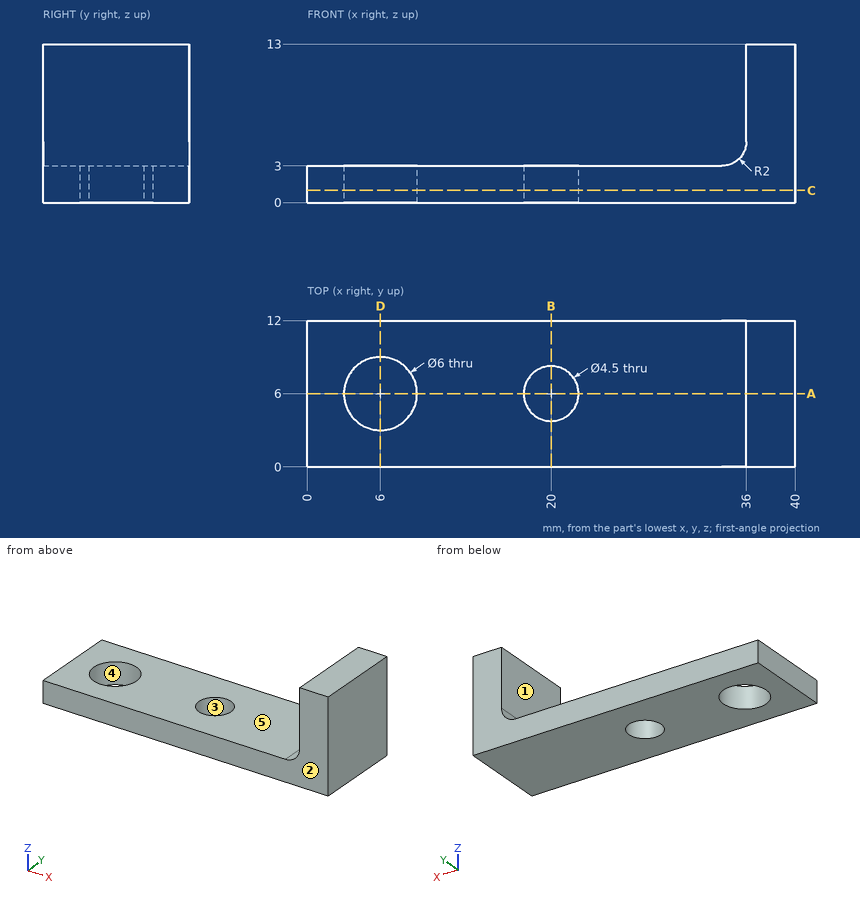
Check sheet for the drawn part. Datum: minimum x, y, z corner. Units: mm. A direction names the side the tool comes from. Coordinates: 2 decimals unless noted, no trailing zeros. Order: outer loops, then holes, each group sorted by start corner. A loop starts at its lowest first (then second) coordinate and runs counter-clockwise, first axis right, second up. Notation, with made-up numbers: M 11,82 L 52,82 A14 cw 52,102 Z; hole C 26,17.25 d10. An arc over 180 degrees is marked long. One line per item, written item: value. Start each with the question number.
Item 1: Sectioned sample at C-C (z = 1). Enter the section's corners in (x, y), then the cut area to 3 significant figures.
Item 2: Gauge pin test, flat ends, axial feed: pin 1 (5 mm diameter, centred on x = 6, y = 6, fed in from -Z); pin 2 (3.5 mm diameter, centred on x = 22.5, y = 7, fed in from +Z); pin 3 (3 mm diameter, centred on x = 27, y = 7.5, fed in from -Z); pin 4 (6.5 mm diameter, centred on y = 8.5, z = 8, fed in from -X). Record the tip position at first contact, or that the pin passes through.
Item 3: Mould release check, pull along X, two halves, no side actions. Record for the marked faces 1, 2 and 3: released by +X, released by -X, zero draft, split by the parting line, or undercut.
Item 4: Access from +Z, -Z, +X, -X, +Y, -Y to the whole of each face (thin tool, end or side, straight path). Record for the marked faces 4 and 5.
Item 5: Scan lines: probe 1 along X at (y, z) = (7.75, 2.5); probe 2 along Z at (x, y) = (33, 3.5); probe 3 along Y at (x, z) = (6, 0.7). Record each from-to range of solid material in increasing order.
Item 6: Sectioned sample at B-B (x = 20). Enter the section's corners in (y, z).
Item 7: Sectioned sample at A-A (y = 6). Enter the section's corners in (x, z), then the cut area to 3 significant figures.
Item 8: Sectioned sample at D-D (x = 6). Enter the section's corners in (y, z).
Conclusion:
1. outline: M 0,0 L 40,0 L 40,12 L 0,12 Z; hole C 6,6 d6; hole C 20,6 d4.5
1. area: 436 mm^2
2. pin 1: passes through
2. pin 2: stops at z = 3
2. pin 3: stops at z = 0
2. pin 4: stops at x = 35.98
3. face 1: released by -X
3. face 2: zero draft
3. face 3: undercut
4. face 4: +Z, -Z
4. face 5: +Z, -X, +Y, -Y
5. probe 1: x = 0 to 3.56, 8.44 to 18.59, 21.41 to 40
5. probe 2: z = 0 to 3
5. probe 3: y = 0 to 3, 9 to 12
6. outline: M 0,0 L 3.75,0 L 3.75,3 L 0,3 Z; M 8.25,0 L 12,0 L 12,3 L 8.25,3 Z
7. outline: M 0,0 L 3,0 L 3,3 L 0,3 Z; M 9,0 L 17.75,0 L 17.75,3 L 9,3 Z; M 22.25,0 L 40,0 L 40,13 L 36,13 L 36,5 A2 cw 34,3 L 22.25,3 Z
7. area: 129 mm^2
8. outline: M 0,0 L 3,0 L 3,3 L 0,3 Z; M 9,0 L 12,0 L 12,3 L 9,3 Z
